from build123d import *

# Parameters (mm, degrees)
CHAMFER1_SIZE = 3


with BuildPart() as part:
    # Sketch1 → Revolve1 (revolve)
    with BuildSketch(Plane.XY, mode=Mode.PRIVATE) as revolve1_sk:
        Polygon((10.25, 0), (20, 0), (20, 40), (16, 40), (16, 45), (8, 45), (8, 31.299038106), (10.25, 30), align=None)
    revolve(revolve1_sk.sketch.rotate(Axis((0, 45, 0), (0, -1, 0)), 90), axis=Axis((0, 45, 0), (0, -1, 0)))

    # Chamfer1
    chamfer1_edges = [part.edges().sort_by_distance(p)[0] for p in [
        (0, 0, -10.25),
    ]]
    chamfer(chamfer1_edges, length=CHAMFER1_SIZE)


solid = part.part
For this review, take the finished solid that the model builds, in its own axes (mm). A direction names the side the tool comes from. Round coordinates to 2 decimals unless told otherwise and drop trailing zeros. Loops run counter-clockwise (first coordinate to the right, second up) from the corner with the lowest first, then second, coordinate; pieces in that order, holes last. Notation, with made-up numbers: (-25.5, 83) - (-0.5, 83) arc R23 cw to (-0.5, 104) - close; hole circle Ø5 at (33.5, 38). An arc over 180 degrees is marked (long way). Use one line per item in the form item = value.
1) Tool access review of faces 1 (the face through (3.926, 16.311, 9.468)), 2 (the face through (-0.88, 20.28, -19.98)): name each direction out of +Z, -Z, +X, -X, +Y, -Y from which nothing blocks a thin tool from reaching the whole face with its end or side.
Solutions:
face_1 = -Y
face_2 = +Y, -Y
2) We need section D-D on y = 29. Write out the cut boundary in (x, z), then the cut area to 3 significant figures.
Solutions:
outline = circle Ø40 at (0, 0); hole circle Ø20.5 at (0, 0)
area = 927 mm2
3) We need section A-A on z = 0. Write out the cut boundary in (x, y), then the cut area to 3 significant figures.
Solutions:
outline = (-20, 0) - (-13.25, 0) - (-10.25, 3) - (-10.25, 30) - (-8, 31.3) - (-8, 45) - (-16, 45) - (-16, 40) - (-20, 40) - close; (8, 31.3) - (10.25, 30) - (10.25, 3) - (13.25, 0) - (20, 0) - (20, 40) - (16, 40) - (16, 45) - (8, 45) - close
area = 893 mm2
4) Clearance check with flat-ended pins moving along their axes: P1, Ø16.5, axis at x = 0, z = 0, coming from the -Y side; P2, Ø10, axis at y = 6.5, z = 14, coming from the -X side; P3, Ø3, axis at y = 16, z = -2.5, coming from the +X side (3 decimals). State where each tip first meets the part, or that it passes through.
Solutions:
P1 = 31.15
P2 = -17.86
P3 = 19.975
5) We need section C-C on y = 41. Write out the cut boundary in (x, z).
Solutions:
outline = circle Ø32 at (0, 0); hole circle Ø16 at (0, 0)
6) Mouldability with a two-part tool opening along X and no side actions: class faces 3 (the face through (-13.43, 40, -8.98)), 4 (the face through (7.81, 38.05, -1.73)), 5 (the face through (15.62, 42.54, -3.47)) as pulls with the +X half, pulls with the -X half, needs draft (parallel to the pull), parting line crosses it, or undercut.
Solutions:
face_3 = needs draft
face_4 = undercut
face_5 = parting line crosses it
7) We need section B-B on x = 0. Write out the cut boundary in (y, z), then the cut area to 3 significant figures.
Solutions:
outline = (0, -20) - (40, -20) - (40, -16) - (45, -16) - (45, -8) - (31.3, -8) - (30, -10.25) - (3, -10.25) - (0, -13.25) - close; (0, 13.25) - (3, 10.25) - (30, 10.25) - (31.3, 8) - (45, 8) - (45, 16) - (40, 16) - (40, 20) - (0, 20) - close
area = 893 mm2
8) Wall thickness on probe 1 along X at (y, z) = (12, 0); probe 2 along X at (y, z) = (34, 0); probe 3 along Z at (x, y) = (-3, 34): over which ranges is each line inside the solid? List them lowest first.
Solutions:
probe_1 = -20 to -10.25, 10.25 to 20
probe_2 = -20 to -8, 8 to 20
probe_3 = -19.77 to -7.42, 7.42 to 19.77
